For this review, use the dimensioned drawing (mm, ordinates from the lowest corner) and the shaded views. Give positions to 0.01 mm unless a question says otherwise; leave off trailing zeros. Loops run counter-clockwise (first coordinate to the right, second up) from the corner with the lowest first, then second, coordinate; pieces in that order, holes last. Notation, with made-up numbers: M -23,-39.75 L -6,-39.75 A31 ccw -6,-3.75 Z; hole C 44.25,87 d1. An arc over 180 degrees is marked long. Return JSON: item names as keys, results as strings.
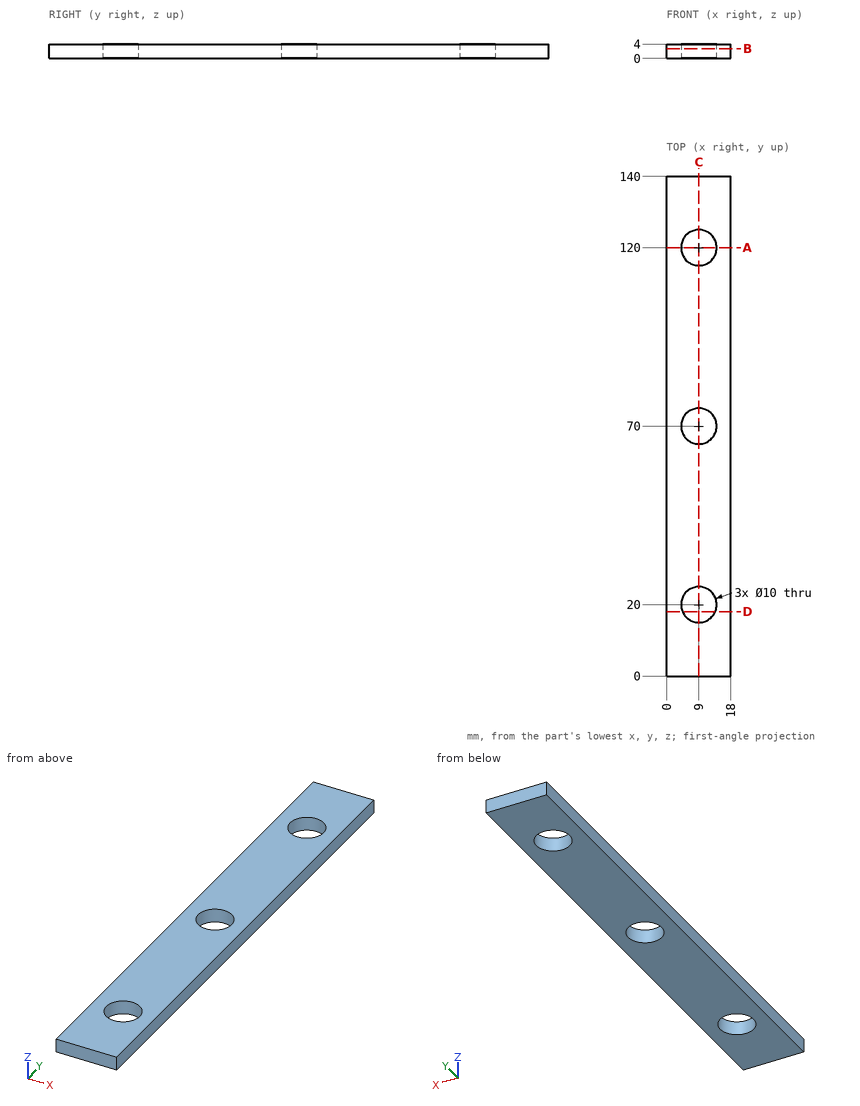
1) Wall thickness on L1, parallel to Y at x = 8.5, z = 3.15; L2, parallel to X at y = 19.5, z = 1.75; L3, parallel to Y at x = 7.5, z = 3.85: over which ranges is each line inside the solid? List them lowest first. Write a range as from..to.
From the geometry:
{"L1": "0..15.03, 24.97..65.03, 74.97..115.03, 124.97..140", "L2": "0..4.03, 13.97..18", "L3": "0..15.23, 24.77..65.23, 74.77..115.23, 124.77..140"}
2) Consider section B-B on z = 2.7. Write out the cut boundary in (x, y), then the cut area to 3 significant figures.
From the geometry:
{"outline": "M 0,0 L 18,0 L 18,140 L 0,140 Z; hole C 9,20 d10; hole C 9,70 d10; hole C 9,120 d10", "area": "2,280 mm²"}
3) Consider section A-A on y = 120. Write out the cut boundary in (x, z).
From the geometry:
{"outline": "M 0,0 L 4,0 L 4,4 L 0,4 Z; M 14,0 L 18,0 L 18,4 L 14,4 Z"}
4) Consider section C-C on x = 9. Write out the cut boundary in (y, z), then the cut area to 3 significant figures.
From the geometry:
{"outline": "M 0,0 L 15,0 L 15,4 L 0,4 Z; M 25,0 L 65,0 L 65,4 L 25,4 Z; M 75,0 L 115,0 L 115,4 L 75,4 Z; M 125,0 L 140,0 L 140,4 L 125,4 Z", "area": "440 mm²"}
5) Consider section D-D on y = 18. Write out the cut boundary in (x, z), then the cut area to 3 significant figures.
From the geometry:
{"outline": "M 0,0 L 4.42,0 L 4.42,4 L 0,4 Z; M 13.58,0 L 18,0 L 18,4 L 13.58,4 Z", "area": "35.3 mm²"}
